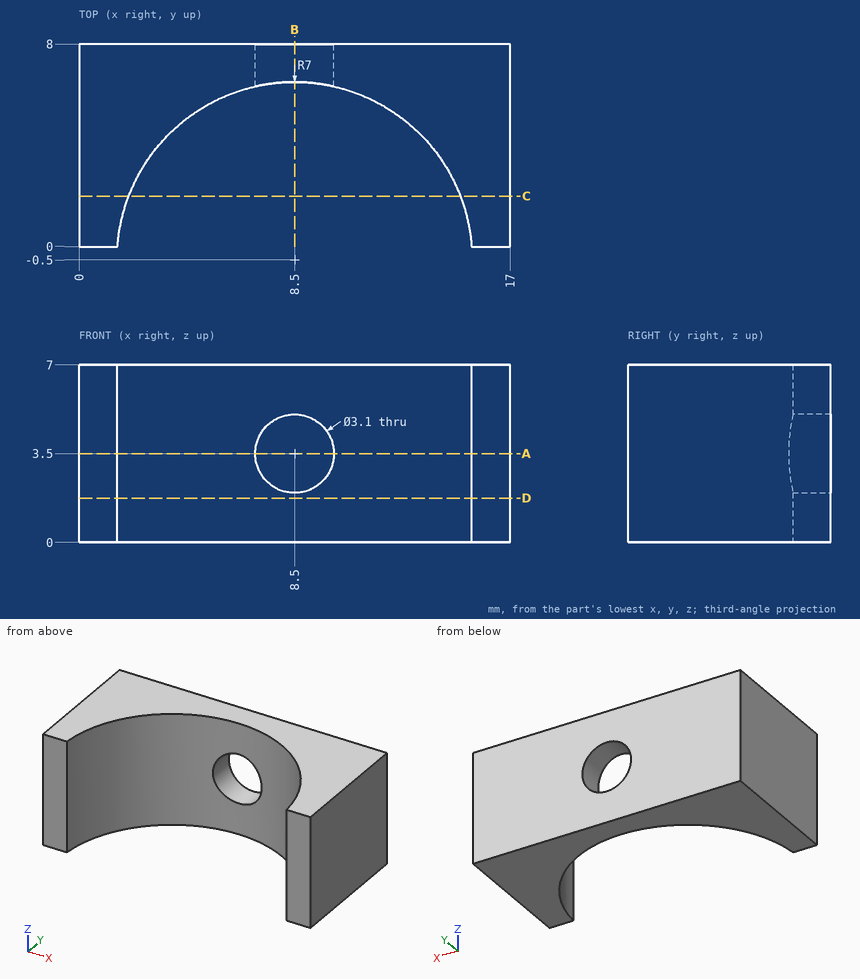
Could you check a few things on this drawing? It's one solid part, dimensions in mm from its lowest x, y, z. Coordinates: 2 decimals unless noted, no trailing zeros. Order: outer loops, then holes, each group sorted by start corner. A loop starts at its lowest first (then second) coordinate and runs counter-clockwise, first axis right, second up. Notation, with made-up numbers: (42.25, 12.25) -> (75.25, 12.25) arc R18 cw to (75.25, 27.25) -> close; hole circle Ø5 at (39.25, 79). An arc over 180 degrees is marked (long way). Answer in a Markdown table with one row per item.
(1) Please list where these lines run through material, in increasing order: probe 1 along X at (y, z) = (7.35, 3.5); probe 2 along Z at (x, y) = (8.5, 7.35); probe 3 along X at (y, z) = (5.75, 2.75).
Answer key:
| item | result |
|---|---|
| probe 1 | 0 to 6.95, 10.05 to 17 |
| probe 2 | 0 to 1.95, 5.05 to 7 |
| probe 3 | 0 to 5.35, 11.65 to 17 |
(2) I want a section at B-B on x = 8.5. List the corners of the cut face in (y, z) for me.
Answer key:
| item | result |
|---|---|
| outline | (6.5, 0) -> (8, 0) -> (8, 1.95) -> (6.5, 1.95) -> close; (6.5, 5.05) -> (8, 5.05) -> (8, 7) -> (6.5, 7) -> close |
(3) I want a section at C-C on y = 2. List the corners of the cut face in (x, z) for me, then the cut area to 3 significant figures.
Answer key:
| item | result |
|---|---|
| outline | (0, 0) -> (1.96, 0) -> (1.96, 7) -> (0, 7) -> close; (15.04, 0) -> (17, 0) -> (17, 7) -> (15.04, 7) -> close |
| area | 27.5 mm^2 |
(4) I want a section at D-D on z = 1.75. List the corners of the cut face in (x, y) for me.
Answer key:
| item | result |
|---|---|
| outline | (0, 0) -> (1.52, 0) arc R7 cw to (15.48, 0) -> (17, 0) -> (17, 8) -> (0, 8) -> close |
(5) I want a section at A-A on z = 3.5. List the corners of the cut face in (x, y) for me, then the cut area to 3 significant figures.
Answer key:
| item | result |
|---|---|
| outline | (0, 0) -> (1.52, 0) arc R7 cw to (6.95, 6.33) -> (6.95, 8) -> (0, 8) -> close; (10.05, 6.33) arc R7 cw to (15.48, 0) -> (17, 0) -> (17, 8) -> (10.05, 8) -> close |
| area | 61.2 mm^2 |
